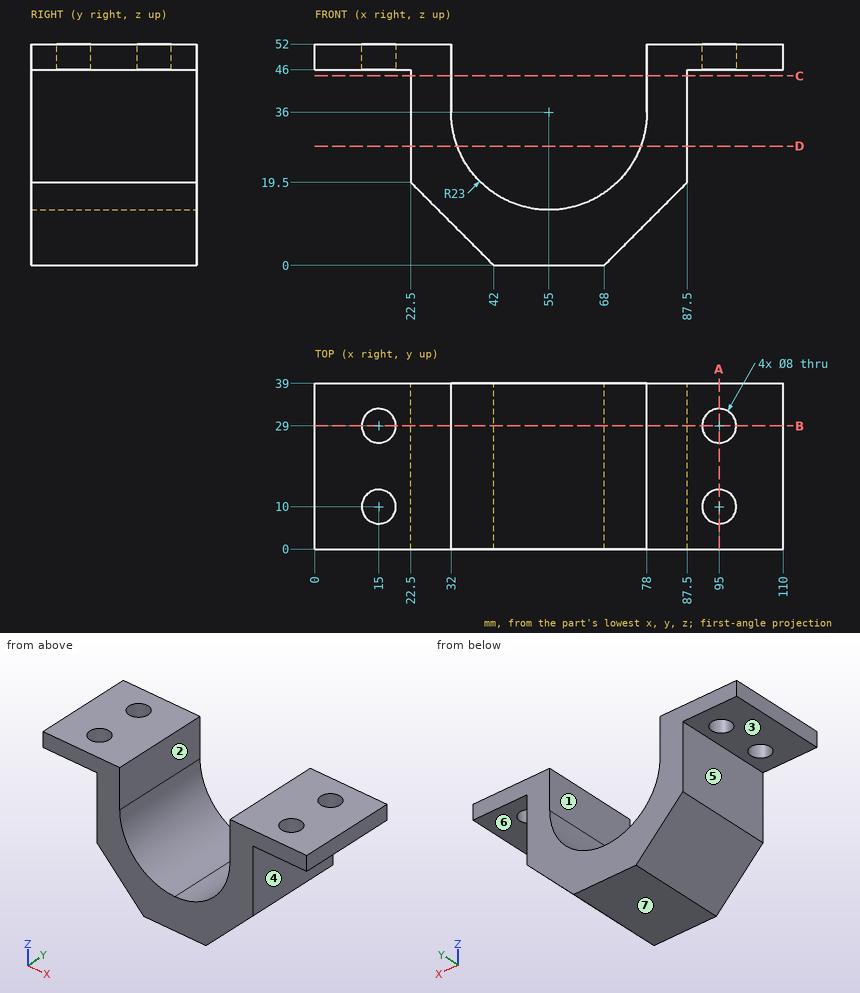
Drawing for the job (mm, zero at the part's lowest x, y, z). A direction names the side the tool comes from. Round coordinates to 2 decimals unless told otherwise and drop trailing zeros. Write each loop counter-clockwise with the first axis right and the second up, starting at its lowest first coordinate (ties: lowest second). Pieces come first, ordered by that corner, then holes.
Item 1: Drop flat-ended pins along their axis: pin 1 Ø13 at (x, y) = (15, 10) entering from -Z; pin 2 Ø6 at (y, z) = (15, 35.5) entering from -X; pin 3 Ø5 at (x, y) = (15, 29) entering from +Z; pin 4 Ø8 at (x, y) = (74, 30.5) entering from -Z. Give the stop position or say it passes through.
Filled in:
pin 1: stops at z = 46
pin 2: stops at x = 22.5
pin 3: passes through
pin 4: stops at z = 2
Item 2: Band-saw the part on D-D on z = 28. Write the cut outline in (x, y).
Filled in:
outline: (22.5, 0) - (33.44, 0) - (33.44, 39) - (22.5, 39) - close; (76.56, 0) - (87.5, 0) - (87.5, 39) - (76.56, 39) - close
Item 3: Tool access for the marked faces 5, 6 and 7: list every direction of +Z, -Z, +X, -X, +Y, -Y with a clear straight run to the whole face (end or side of a thin tool).
Filled in:
face 5: -Z, -X, +Y, -Y
face 6: -Z, +X, +Y, -Y
face 7: -Z, +X, -X, +Y, -Y
Item 4: Mould opens along X. For the marked faces 1, 2, 3 and 4 say: released by +X, released by -X, zero draft, split by the parting line, or undercut.
Filled in:
face 1: undercut
face 2: undercut
face 3: zero draft
face 4: released by +X
Item 5: Drill centre lines: L1, parallel to Y at x = 15, z = 49; L2, parallel to X at y = 17.5, z = 37; L3, parallel to X at y = 33, z = 20.5. Where is each one in solid material? Low to high.
Filled in:
L1: y = 0 to 6, 14 to 25, 33 to 39
L2: x = 22.5 to 32, 78 to 87.5
L3: x = 22.5 to 38.01, 71.99 to 87.5
Item 6: Band-saw the part on A-A on x = 95. Write the cut outline in (y, z), then the cut area to 3 significant figures.
Filled in:
outline: (0, 46) - (6, 46) - (6, 52) - (0, 52) - close; (14, 46) - (25, 46) - (25, 52) - (14, 52) - close; (33, 46) - (39, 46) - (39, 52) - (33, 52) - close
area: 138 mm2
Item 7: Band-saw the part on C-C on z = 44.5. Write the cut outline in (x, y).
Filled in:
outline: (22.5, 0) - (32, 0) - (32, 39) - (22.5, 39) - close; (78, 0) - (87.5, 0) - (87.5, 39) - (78, 39) - close
Item 8: Band-saw the part on B-B on y = 29. Write the cut outline in (x, z), then the cut area to 3 significant figures.
Filled in:
outline: (0, 46) - (11, 46) - (11, 52) - (0, 52) - close; (19, 46) - (22.5, 46) - (22.5, 19.5) - (42, 0) - (68, 0) - (87.5, 19.5) - (87.5, 46) - (91, 46) - (91, 52) - (78, 52) - (78, 36) arc R23 cw to (32, 36) - (32, 52) - (19, 52) - close; (99, 46) - (110, 46) - (110, 52) - (99, 52) - close
area: 1,610 mm2
